Print and shaded views of the part. All mm, measured from the part's lowest x, y and z. Round coordinates to 2 decimals unless told otherwise and drop trailing zeros. Loops run counter-clockwise (first coordinate to the right, second up) from the corner with the lowest first, then second, coordinate; pieces in that order, holes last. Notation, with made-up numbers: (27, 54) - (47, 54) arc R21 ccw to (47, 82) - close; hole circle Ø6 at (-18, 32.5). An arc over 180 degrees is marked (long way). Put each result on its own line as item: value. Start each with the question number.
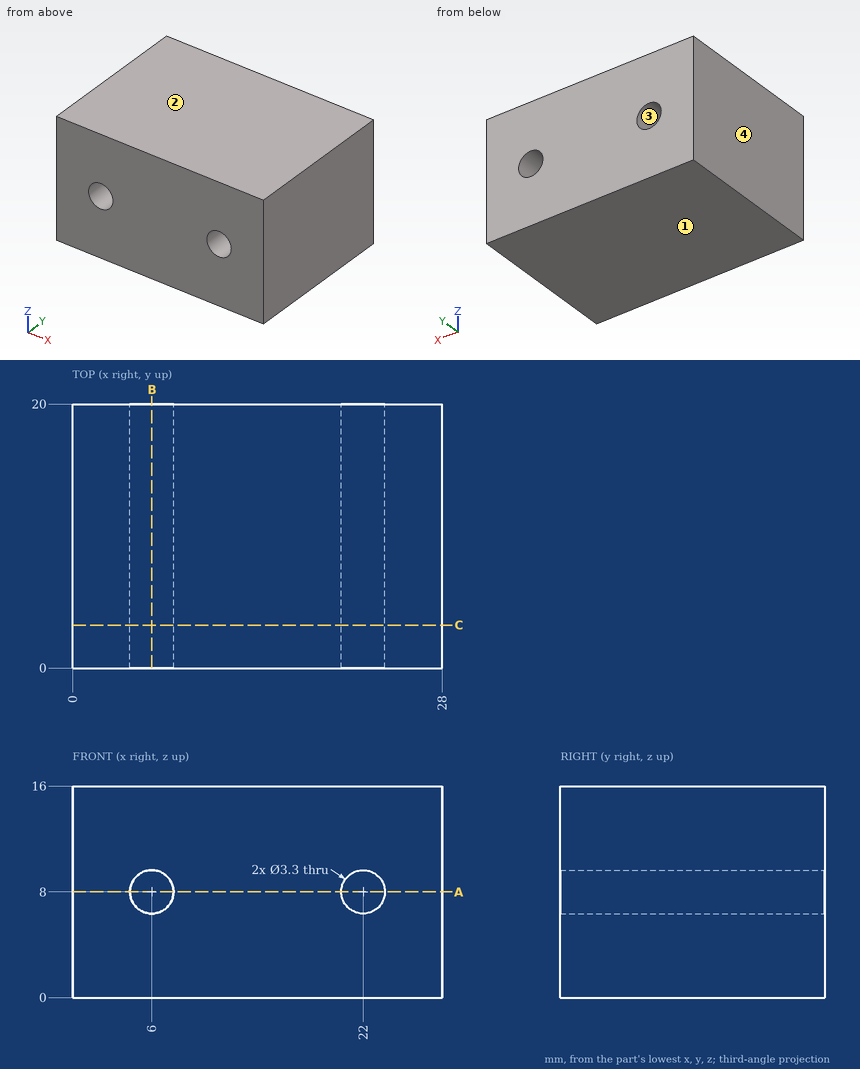
Item 1: Drop a flat-ended pin along its axis: pin 1 Ø2.5 at (x, z) = (6, 8) entering from -Y. Give the stop position or say it passes through.
Item 2: Slice it at C-C (y = 3.25). Give the cut face in (x, z), plus the area to 3 significant figures.
Item 3: Drill centre lines: probe 1 along X at (y, z) = (9.75, 8); probe 2 along Z at (x, y) = (6, 5.75). Where is each one in solid material? Low to high. Write a range as [from, to].
Item 4: Two-plate mould, pull along Z, no slides. Class the marked faces 1, 2, 3 and 4: pulls with the +Z half, pulls with the -Z half, needs draft (parallel to the pull), parting line crosses it, or undercut.
Item 5: Slice it at B-B (x = 6). Give the cut face in (y, z), plus the area to 3 significant figures.
Item 6: Slice it at A-A (z = 8). Give the cut face in (x, y), plus the area to 3 significant figures.
Computed values:
1. pin 1: passes through
2. outline: (0, 0) - (28, 0) - (28, 16) - (0, 16) - close; hole circle Ø3.3 at (6, 8); hole circle Ø3.3 at (22, 8)
2. area: 431 mm^2
3. probe 1: x = [0, 4.35], [7.65, 20.35], [23.65, 28]
3. probe 2: z = [0, 6.35], [9.65, 16]
4. face 1: pulls with the -Z half
4. face 2: pulls with the +Z half
4. face 3: undercut
4. face 4: needs draft
5. outline: (0, 0) - (20, 0) - (20, 6.35) - (0, 6.35) - close; (0, 9.65) - (20, 9.65) - (20, 16) - (0, 16) - close
5. area: 254 mm^2
6. outline: (0, 0) - (4.35, 0) - (4.35, 20) - (0, 20) - close; (7.65, 0) - (20.35, 0) - (20.35, 20) - (7.65, 20) - close; (23.65, 0) - (28, 0) - (28, 20) - (23.65, 20) - close
6. area: 428 mm^2
